Read the model definition and answer for the solid it produces. Units are mm, in the model's axes. A direction names the side the tool comes from. Coordinates: 2 decimals unless noted, no trailing zeros. Order: outer loops, then holes, each group sorted by start corner. A loop starts at its lowest first (then second) coordinate and runs counter-clockwise, first axis right, second up. Notation, with made-up numbers: (8.5, 81) - (27.5, 81) arc R11 ccw to (27.5, 88) - close; hole circle Ø10 at (81.5, 67). An arc over 180 degrees is marked (long way). Use one line per item in the form item = value.
```python
from build123d import *

# Parameters (mm, degrees)
SKETCH1_W           = 60
SKETCH1_H           = 60
BOSS_EXTRUDE1_DEPTH = 20
BOSS_EXTRUDE2_DEPTH = 70
SKETCH8_R           = 8.25
CUT_EXTRUDE5_DEPTH  = 8


with BuildPart() as part:
    # Sketch1 → Boss-Extrude1 (new body)
    with BuildSketch(Plane(origin=(0, 0, 0), x_dir=(1, 0, 0), z_dir=(0, 1, 0))):
        Rectangle(SKETCH1_W, SKETCH1_H)
    extrude(amount=BOSS_EXTRUDE1_DEPTH)

    # Sketch2 → Boss-Extrude2 (add)
    with BuildSketch(Plane(origin=(30, 0, 0), x_dir=(0, 0, -1), z_dir=(1, 0, 0))):
        Polygon((30, 20), (30, 0), (30, -7), (-12, -22), (-30, -22), (-30, 20), align=None)
    extrude(amount=-BOSS_EXTRUDE2_DEPTH)

    # Sketch8 → Cut-Extrude5 (cut)
    with BuildSketch(Plane.XY.offset(30)):
        with Locations((0, -9)):
            Circle(SKETCH8_R)
    extrude(amount=-CUT_EXTRUDE5_DEPTH, mode=Mode.SUBTRACT)


solid = part.part
```
(1) Which of the six approach directions +Z, -Z, +X, -X, +Y, -Y give full straight-line access (tool end or side, diameter ignored) to faces 4 (the flat face through (-5, 20, 0)), 5 (the flat face through (0, -9, 22))?
Answer list:
face_4 = +Z, -Z, +X, -X, +Y
face_5 = +Z
(2) Section B-B, the plane x = 0 is taken. Write down the section's boundary in (y, z), then the cut area to 3 significant figures.
Answer list:
outline = (-22, 12) - (-7, -30) - (20, -30) - (20, 30) - (-0.75, 30) - (-0.75, 22) - (-17.25, 22) - (-17.25, 30) - (-22, 30) - close
area = 2,070 mm2
(3) Section A-A, the plane y = -9 is taken. Write down the section's boundary in (x, z).
Answer list:
outline = (-40, -24.4) - (30, -24.4) - (30, 30) - (8.25, 30) - (8.25, 22) - (-8.25, 22) - (-8.25, 30) - (-40, 30) - close
(4) The mould has two halves that part along Y. Classify faces 1 (the cylindrical face through (3.807, -16.319, 26.056)), 2 (the flat face through (-5, -1, 30)), 3 (the flat face through (-5, -22, 21)): +Y half, -Y half, draft (parallel to the pull), parting line (faces both ways), or undercut.
Answer list:
face_1 = undercut
face_2 = draft
face_3 = -Y half
(5) Straight lines are drawn through the part: L1, parallel to Y at x = 0, z = 24.5; L2, parallel to Y at x = -7, z = -26; L3, parallel to Y at x = -19, z = -24.5. For each, find the intervals that lie inside material, in ascending order.
Answer list:
L1 = -22 to -17.25, -0.75 to 20
L2 = -8.43 to 20
L3 = -8.96 to 20
(6) Section D-D, the plane x = -10 is taken. Write down the section's boundary in (y, z).
Answer list:
outline = (-22, 12) - (-7, -30) - (20, -30) - (20, 30) - (-22, 30) - close
(7) Section C-C, the plane z = -16 is taken. Write down the section's boundary in (x, y).
Answer list:
outline = (-40, -12) - (30, -12) - (30, 20) - (-40, 20) - close
